Verification items for the finished model (mm, model axes). A direction names the side the tool comes from. Coordinates: 2 decimals unless noted, no trailing zeros. Write each loop counter-clockwise with the first axis right and the second up, starting at its lowest first coordinate (ties: lowest second). Pieces come first, ordered by that corner, then holes. Notation, with made-up numbers: (1, -19.5) -> (48, -19.5) arc R25 ccw to (48, 6.5) -> close; hole circle Ø9 at (25, 42). An arc over 180 degrees is marked (long way). Write item = value, one per line. Start each with the question number.
(1) Mould release check, pull along X, two halves, no side actions. Record for faces 6 (the face through (15.78, 3.32, -0.74)), 7 (the face through (0.14, -9.64, 0.2)), 8 (the face through (5, 4.2, -4.5)): released by +X, released by -X, zero draft, split by the parting line, or undercut.
(2) Material ranges on probe 1 along Z at (x, y) = (21.75, -0.25); probe 2 along X at (y, z) = (-4.75, 0.25); probe 3 along X at (y, z) = (-5, 5.75), recorded low to high. Write a range as [from, to].
(3) Section check D-D (x = 10). Record the cut outline in (y, z), plus the area to 3 significant figures.
(4) Gauge pin test, flat ends, axial feed: pin 1 Ø8 at (y, z) = (-2, -7.5) entering from +X; pin 2 Ø6 at (x, z) = (14.5, 7.5) entering from -Y; pin 3 Ø5 at (x, y) = (9, 4) entering from +Z. Record the tip position at first contact, or that the pin passes through.
(5) Section check C-C (x = 22.5). Record the cut outline in (y, z).
(6) Section check B-B (z = 0). Record the cut outline in (x, y), plus the area to 3 significant figures.
(7) Set-up check for faces 1 (the face through (15.5, 4, 0)), 2 (the face through (1, -1, 0)), 3 (the face through (0, -4, 0)), 4 (the face through (27, 0, 0)), 5 (the face through (21.593, 3.905, -0.867)): record each of +Z, -Z, +X, -X, +Y, -Y from which the full face is reachable in a straight line by a thin tool's end or side.
(8) Section check A-A (y = 0). Record the cut outline in (x, z).
```python
from build123d import *

# Parameters (mm, degrees)
CHAMFER1_SIZE           = 0.5
CUT_EXTRUDE1_DEPTH      = 31.479501308
CUT_EXTRUDE1_DEPTH_BACK = 31.479501308
SKETCH3_W               = 2.5
SKETCH3_H               = 2
FILLET1_R               = 0.25


with BuildPart() as part:
    # Sketch2 → Revolve1 (revolve)
    with BuildSketch(Plane.XY, mode=Mode.PRIVATE) as revolve1_sk:
        Polygon((0, 0), (0, 10), (5, 10), (5, 6), (15.5, 6), (15.5, 4), (15.5, 3.4), (16.05, 3.4), (16.65, 4), (26.4, 4), (27, 3.4), (27, 0), align=None)
    revolve(revolve1_sk.sketch.rotate(Axis((0, 0, 0), (1, 0, 0)), 90), axis=Axis((0, 0, 0), (1, 0, 0)))

    # Chamfer1
    chamfer1_edges = [part.edges().sort_by_distance(p)[0] for p in [
        (0, 0, -10),
    ]]
    chamfer(chamfer1_edges, length=CHAMFER1_SIZE)

    # Sketch3 → Cut-Extrude1 (cut, two sides: drawn at the far end of the back side and taken through both)
    with BuildSketch(Plane.XY.offset(-CUT_EXTRUDE1_DEPTH_BACK)):
        with Locations((1.25, 0)):
            Rectangle(SKETCH3_W, SKETCH3_H)
    extrude(amount=CUT_EXTRUDE1_DEPTH + CUT_EXTRUDE1_DEPTH_BACK, mode=Mode.SUBTRACT)

    # Fillet1
    fillet1_edges = [part.edges().sort_by_distance(p)[0] for p in [
        (15.5, 0, -6),
        (5, 0, -10),
    ]]
    fillet(fillet1_edges, radius=FILLET1_R)


solid = part.part
```
Response:
q1.face_6 = undercut
q1.face_7 = released by -X
q1.face_8 = released by +X
q2.probe_1 = [-3.99, 3.99]
q2.probe_2 = [0, 15.5]
q2.probe_3 = [0, 5]
q3.outline = circle Ø12 at (0, 0)
q3.area = 113 mm2
q4.pin_1 = 26.64
q4.pin_2 = -3.97
q4.pin_3 = 5.81
q5.outline = circle Ø8 at (0, 0)
q6.outline = (0, -9.5) -> (0.5, -10) -> (4.75, -10) arc R0.25 ccw to (5, -9.75) -> (5, -6) -> (15.25, -6) arc R0.25 ccw to (15.5, -5.75) -> (15.5, -3.4) -> (16.05, -3.4) -> (16.65, -4) -> (26.4, -4) -> (27, -3.4) -> (27, 3.4) -> (26.4, 4) -> (16.65, 4) -> (16.05, 3.4) -> (15.5, 3.4) -> (15.5, 5.75) arc R0.25 ccw to (15.25, 6) -> (5, 6) -> (5, 9.75) arc R0.25 ccw to (4.75, 10) -> (0.5, 10) -> (0, 9.5) -> (0, 1) -> (2.5, 1) -> (2.5, -1) -> (0, -1) -> close
q6.area = 311 mm2
q7.face_1 = none
q7.face_2 = +Z, -Z, -X
q7.face_3 = +Z, -Z, -X, +Y, -Y
q7.face_4 = +Z, -Z, +X, +Y, -Y
q7.face_5 = +X
q8.outline = (2.5, -10) -> (4.75, -10) arc R0.25 ccw to (5, -9.75) -> (5, -6) -> (15.25, -6) arc R0.25 ccw to (15.5, -5.75) -> (15.5, -3.4) -> (16.05, -3.4) -> (16.65, -4) -> (26.4, -4) -> (27, -3.4) -> (27, 3.4) -> (26.4, 4) -> (16.65, 4) -> (16.05, 3.4) -> (15.5, 3.4) -> (15.5, 5.75) arc R0.25 ccw to (15.25, 6) -> (5, 6) -> (5, 9.75) arc R0.25 ccw to (4.75, 10) -> (2.5, 10) -> close
